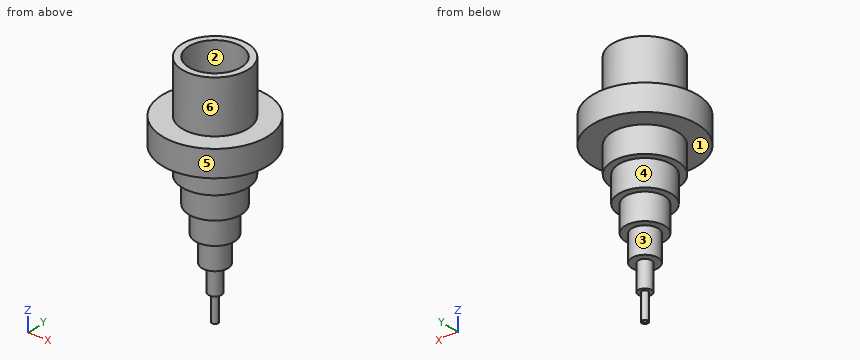
```python
from build123d import *

# Parameters (mm, degrees)
FLANGE_PROFILE_80_R    = 40
FLANGE_80_DEPTH        = 20
STEP_50_PROFILE_R      = 25
SHAFT_STEP_50_DEPTH    = 40
STEP_40_PROFILE_R      = 20
SHAFT_STEP_40_DEPTH    = 60
STEP_30_PROFILE_R      = 15
SHAFT_STEP_30_DEPTH    = 80
STEP_20_PROFILE_R      = 10
SHAFT_STEP_20_DEPTH    = 100
STEP_10_PROFILE_R      = 5
SHAFT_STEP_10_DEPTH    = 120
TIP_PIN_5_PROFILE_R    = 2.5
TIP_PIN_5_DEPTH        = 140
HUB_START              = 40
HUB_50_PROFILE_R       = 25
HUB_50_DEPTH           = 40
HUB_BORE_40_PROFILE_R  = 20
HUB_BORE_40_DEPTH      = 40
AXIAL_BORE_3_PROFILE_R = 1.5
AXIAL_BORE_3_DEPTH     = 140


with BuildPart() as part:
    # Flange Profile Ø80 → Flange Ø80 (new body)
    with BuildSketch(Plane.XY):
        Circle(FLANGE_PROFILE_80_R)
    extrude(amount=-FLANGE_80_DEPTH)

    # Step Ø50 Profile → Shaft Step Ø50 (add)
    with BuildSketch(Plane.XY):
        Circle(STEP_50_PROFILE_R)
    extrude(amount=-SHAFT_STEP_50_DEPTH)

    # Step Ø40 Profile → Shaft Step Ø40 (add)
    with BuildSketch(Plane.XY):
        Circle(STEP_40_PROFILE_R)
    extrude(amount=-SHAFT_STEP_40_DEPTH)

    # Step Ø30 Profile → Shaft Step Ø30 (add)
    with BuildSketch(Plane.XY):
        Circle(STEP_30_PROFILE_R)
    extrude(amount=-SHAFT_STEP_30_DEPTH)

    # Step Ø20 Profile → Shaft Step Ø20 (add)
    with BuildSketch(Plane.XY):
        Circle(STEP_20_PROFILE_R)
    extrude(amount=-SHAFT_STEP_20_DEPTH)

    # Step Ø10 Profile → Shaft Step Ø10 (add)
    with BuildSketch(Plane.XY):
        Circle(STEP_10_PROFILE_R)
    extrude(amount=-SHAFT_STEP_10_DEPTH)

    # Tip Pin Ø5 Profile → Tip Pin Ø5 (add)
    with BuildSketch(Plane.XY):
        Circle(TIP_PIN_5_PROFILE_R)
    extrude(amount=-TIP_PIN_5_DEPTH)

    # Hub Ø50 Profile → Hub Ø50 (add)
    with BuildSketch(Plane.XY.offset(HUB_START)):
        Circle(HUB_50_PROFILE_R)
    extrude(amount=-HUB_50_DEPTH)

    # Hub Bore Ø40 Profile → Hub Bore Ø40 (cut)
    with BuildSketch(Plane.XY.offset(40)):
        Circle(HUB_BORE_40_PROFILE_R)
    extrude(amount=-HUB_BORE_40_DEPTH, mode=Mode.SUBTRACT)

    # Axial Bore Ø3 Profile → Axial Bore Ø3 (cut)
    with BuildSketch(Plane.XY):
        Circle(AXIAL_BORE_3_PROFILE_R)
    extrude(amount=-AXIAL_BORE_3_DEPTH, mode=Mode.SUBTRACT)


solid = part.part
```
CAD build for the part. Positions are in the model's coordinates, mm. Face numbers are marked on the shaded views. A direction names the side the tool comes from. Round coordinates to 2 decimals unless told otherwise and drop trailing zeros. Loops run counter-clockwise (first coordinate to the right, second up) from the corner with the lowest first, then second, coordinate; pieces in that order, holes last. Notation, with made-up numbers: M 48,45 L 85,45 A25 cw 85,81 Z; hole C 2,46 d7. An arc over 180 degrees is marked long. Return JSON: item names as keys, results as strings. Group by question number.
(1) Mould opens along X. For the marked faces 1, 2 and 3 say: +X half, -X half, draft (parallel to the pull), parting line (faces both ways), or undercut.
(2) Saw through at A-A, the plane z = -37.5. List the corners of the cut face in (x, y), and give its area (3 significant figures).
(3) Saw through at C-C, the plane z = -96. List the corners of the cut face in (x, y).
(4) Saw through at D-D, the plane x = -8. List the corners of the cut face in (y, z).
(5) Drop flat-ended pins along their axis: P1, Ø8, axis at y = 12, z = -82.5, coming from the +X side; P2, Ø5, axis at x = 0, z = -49.5, coming from the -Y side; P3, Ø10, axis at x = 12, z = 13, coming from the +Y side. Give the stop position or say it passes through.
(6) Tool access for the marked faces 4, 5 and 6: list every direction of +Z, -Z, +X, -X, +Y, -Y with a clear straight run to the whole face (end or side of a thin tool).
(7) Saw through at B-B, the plane x = -18. List the corners of the cut face in (y, z), and give its area (3 significant figures).
(8) Wall check: probe 1 along Y at (x, z) = (0, -102); probe 2 along Y at (x, z) = (0, -91); probe 3 along Z at (x, y) = (24, 5). Give the ranges that are in metal, low to high. Write a range as [from, to].
Answer list:
{
 "1": {"face 1": "draft", "face 2": "undercut", "face 3": "parting line"},
 "2": {"outline": "C 0,0 d50; hole C 0,0 d3", "area": "1,960 mm2"},
 "3": {"outline": "C 0,0 d20; hole C 0,0 d3"},
 "4": {"outline": "M -39.19,-20 L -23.69,-20 L -23.69,-40 L -18.33,-40 L -18.33,-60 L -12.69,-60 L -12.69,-80 L -6,-80 L -6,-100 L 6,-100 L 6,-80 L 12.69,-80 L 12.69,-60 L 18.33,-60 L 18.33,-40 L 23.69,-40 L 23.69,-20 L 39.19,-20 L 39.19,0 L 23.69,0 L 23.69,40 L 18.33,40 L 18.33,0 L -18.33,0 L -18.33,40 L -23.69,40 L -23.69,0 L -39.19,0 Z"},
 "5": {"P1": "x = 12.09", "P2": "y = -20", "P3": "y = 24"},
 "6": {"face 4": "-Z", "face 5": "+Z, -Z", "face 6": "+Z"},
 "7": {"outline": "M -35.72,-20 L -17.35,-20 L -17.35,-40 L -8.72,-40 L -8.72,-60 L 8.72,-60 L 8.72,-40 L 17.35,-40 L 17.35,-20 L 35.72,-20 L 35.72,0 L 17.35,0 L 17.35,40 L 8.72,40 L 8.72,0 L -8.72,0 L -8.72,40 L -17.35,40 L -17.35,0 L -35.72,0 Z", "area": "3,160 mm2"},
 "8": {"probe 1": "[-5, -1.5], [1.5, 5]", "probe 2": "[-10, -1.5], [1.5, 10]", "probe 3": "[-40, 40]"}
}
